Verification items for the finished model (mm, model axes). Give positions to 0.01 mm unless a question says otherwise; leave off trailing zeros. Order: outer loops, then holes, each group sorted by start corner. A loop starts at its lowest first (then second) coordinate and runs counter-clockwise, first axis right, second up.
from build123d import *


with BuildPart() as part:
    # Sketch1 → Revolve1 (revolve)
    with BuildSketch(Plane(origin=(0, 0, 0), x_dir=(0, 0, -1), z_dir=(1, 0, 0))):
        Polygon((0.45, 16), (0.875, 16), (0.875, 50), (0.45, 50), (0.45, 67), (0, 67), (0, -1.75), (0.45, -1.75), align=None)
    revolve(axis=Axis((0, -4.379065135, 0), (0, 1, 0)))


solid = part.part
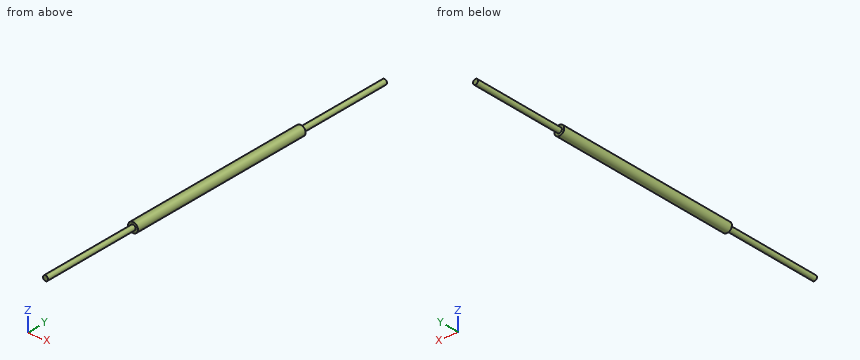
(1) Section check D-D, the plane y = 14.5. Enter the section's corners in (x, z), then the cut area to 3 significant figures.
Solved:
outline: circle Ø0.9 at (0, 0)
area: 0.636 mm2
(2) Section check C-C, the plane y = 26.5. Enter the section's corners in (x, z) (3 decimals).
Solved:
outline: circle Ø1.75 at (0, 0)
(3) Section check B-B, the plane z = 0. Enter the section's corners in (x, y) (3 decimals), then the cut area to 3 significant figures.
Solved:
outline: (-0.875, 16) - (-0.45, 16) - (-0.45, -1.75) - (0.45, -1.75) - (0.45, 16) - (0.875, 16) - (0.875, 50) - (0.45, 50) - (0.45, 67) - (-0.45, 67) - (-0.45, 50) - (-0.875, 50) - close
area: 90.8 mm2
(4) Section check A-A, the plane x = 0. Enter the section's corners in (y, z) (3 decimals).
Solved:
outline: (-1.75, -0.45) - (16, -0.45) - (16, -0.875) - (50, -0.875) - (50, -0.45) - (67, -0.45) - (67, 0.45) - (50, 0.45) - (50, 0.875) - (16, 0.875) - (16, 0.45) - (-1.75, 0.45) - close
(5) Scan lines: line 1 (Y direction, x = -0.35, z = -0.6); line 2 (Z direction, x = 0.75, y = 35). Record each from-to range of solid material in increasing order.
Solved:
line 1: y = 16 to 50
line 2: z = -0.45 to 0.45
